Check sheet for the drawn part. Datum: minimum x, y, z corner. Units: mm. A direction names the side the tool comes from. Give positions to 0.01 mm unless a question says otherwise; leave off trailing zeros. Write each loop counter-clockwise with the first axis right and the second up, starting at its lowest first coordinate (ties: lowest second). Pieces come first, ordered by that corner, then holes.
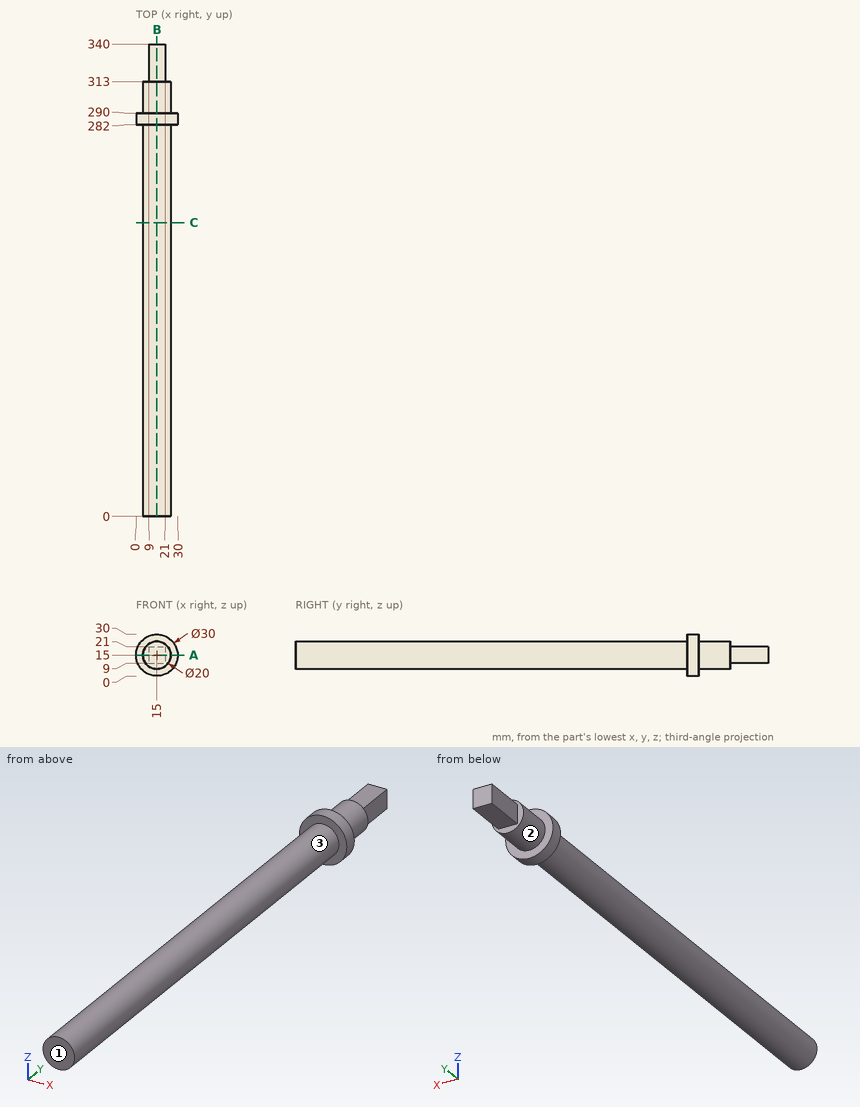
1) Scan lines: L1, parallel to Y at x = 20.5, z = 26; L2, parallel to Y at x = 10, z = 22; L3, parallel to X at y = 246, z = 23. Record each from-to range of solid material in increasing order.
2) Sectioned sample at B-B on x = 15. Record the boundary of the cut face in (y, z), then the cut area to 3 significant figures.
3) Access from +Z, -Z, +X, -X, +Y, -Y to the whole of each face (thin tool, end or side, straight path). Record for the marked faces 1, 2 and 3.
4) Gauge pin test, flat ends, axial feed: pin 1 (12 mm diameter, centred on x = 9.5, y = 296.5, fed in from +Z); pin 2 (3.5 mm diameter, centred on y = 324, z = 16.5, fed in from +X); pin 3 (10 mm diameter, centred on x = 11, y = 78.5, fed in from -Z). Record the tip position at first contact, or that the pin passes through.
5) Sectioned sample at A-A on z = 15. Record the boundary of the cut face in (x, y), then the cut area to 3 significant figures.
6) Sectioned sample at C-C on y = 211.5. Record the boundary of the cut face in (x, z).
Answers below:
1. L1: y = 282 to 290
1. L2: y = 0 to 313
1. L3: x = 9 to 21
2. outline: (0, 5) - (282, 5) - (282, 0) - (290, 0) - (290, 5) - (313, 5) - (313, 9) - (340, 9) - (340, 21) - (313, 21) - (313, 25) - (290, 25) - (290, 30) - (282, 30) - (282, 25) - (0, 25) - close
2. area: 6,660 mm2
3. face 1: +Z, -Z, +X, -X, -Y
3. face 2: +Y
3. face 3: -Y
4. pin 1: stops at z = 25
4. pin 2: stops at x = 21
4. pin 3: stops at z = 5
5. outline: (0, 282) - (5, 282) - (5, 0) - (25, 0) - (25, 282) - (30, 282) - (30, 290) - (25, 290) - (25, 313) - (21, 313) - (21, 340) - (9, 340) - (9, 313) - (5, 313) - (5, 290) - (0, 290) - close
5. area: 6,660 mm2
6. outline: circle Ø20 at (15, 15)
